from build123d import *

# Parameters (mm, degrees)
SKETCH_1_R      = 12
SKETCH_1_R_2    = 6
EXTRUDE_1_DEPTH = 6
CHAMFER_1_SIZE  = 0.2


with BuildPart() as part:
    # 草图1 → 拉伸1 (new body)
    with BuildSketch(Plane(origin=(0, 0, 0), x_dir=(1, 0, 0), z_dir=(0, 1, 0))):
        with Locations(Location((0, 0, 0), (0, 0, 270))):
            Circle(SKETCH_1_R)
        with Locations(Location((0, 0, 0), (0, 0, 270))):
            Circle(SKETCH_1_R_2, mode=Mode.SUBTRACT)
    extrude(amount=EXTRUDE_1_DEPTH)

    # 倒角1
    chamfer_1_edges = [part.edges().sort_by_distance(p)[0] for p in [
        (0, 0, -12),
        (0, 6, -12),
        (0, 0, -6),
        (0, 6, -6),
    ]]
    chamfer(chamfer_1_edges, length=CHAMFER_1_SIZE)


solid = part.part
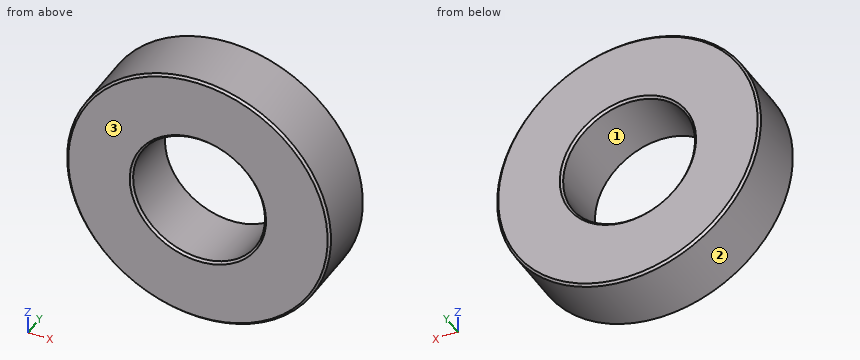
Source: CAD feature listing. Evaluate the final solid. Frame: model axes, mm. Face numbers are marked on the shaded views. Round coordinates to 2 decimals unless told otherwise and drop trailing zeros. Order: outer loops, then holes, each group sorted by start corner. A loop starts at its lowest first (then second) coordinate and runs counter-clockwise, first axis right, second up. Notation, with made-up numbers: (-6.75, 17.25) - (7.25, 17.25) arc R19 ccw to (7.25, 38.25) - close; hole circle Ø11 at (0, -7). An arc over 180 degrees is marked (long way). Use a Markdown table: item, result. Add a question column.
1. First-contact query: pin 1 (2 mm diameter, centred on y = 1, z = -1.5, fed in from +X). Flat tip, straight axial feed; report the tip coordinate or a pass-through.
2. Mould query, pull axis Z, two halves, no side actions, for the marked faces 1, 2 and 3. Classes: +Z half, -Z half, draft (parallel to the pull), parting line (faces both ways), or undercut.
3. Line query: probe 1 along X at (y, z) = (4.7, 0); probe 2 along X at (y, z) = (3.15, -5); probe 3 along Z at (x, y) = (1, 0.5). Output: solid intervals per line, ascending.
4. Section query C-C (y = 1.75). Return the cut outline in (x, z), then the cut area to 3 significant figures.
5. Section query B-B (z = 0). Return the cut outline in (x, y).
6. Section query A-A (x = 0). Return the cut outline in (y, z), then the cut area to 3 significant figures.
Derived:
| question | item | result |
|---|---|---|
| 1 | pin 1 | x = 11.99 |
| 2 | face 1 | undercut |
| 2 | face 2 | parting line |
| 2 | face 3 | draft |
| 3 | probe 1 | -12 to -6, 6 to 12 |
| 3 | probe 2 | -10.91 to -3.32, 3.32 to 10.91 |
| 3 | probe 3 | -11.96 to -5.92, 5.92 to 11.96 |
| 4 | outline | circle Ø24 at (0, 0); hole circle Ø12 at (0, 0) |
| 4 | area | 339 mm2 |
| 5 | outline | (-12, 0.2) - (-11.8, 0) - (-6.2, 0) - (-6, 0.2) - (-6, 5.8) - (-6.2, 6) - (-11.8, 6) - (-12, 5.8) - close; (6, 0.2) - (6.2, 0) - (11.8, 0) - (12, 0.2) - (12, 5.8) - (11.8, 6) - (6.2, 6) - (6, 5.8) - close |
| 6 | outline | (0, -11.8) - (0.2, -12) - (5.8, -12) - (6, -11.8) - (6, -6.2) - (5.8, -6) - (0.2, -6) - (0, -6.2) - close; (0, 6.2) - (0.2, 6) - (5.8, 6) - (6, 6.2) - (6, 11.8) - (5.8, 12) - (0.2, 12) - (0, 11.8) - close |
| 6 | area | 71.8 mm2 |
